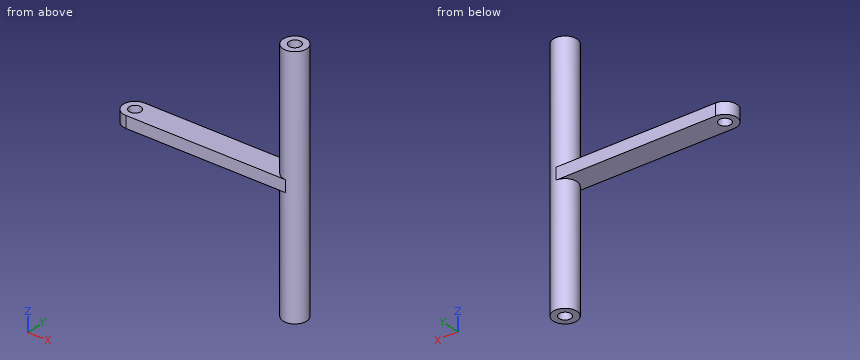
from build123d import *

# Parameters (mm, degrees)
SKETCH_1_R               = 5
SKETCH_1_R_2             = 4.376095709
EXTRUDE_1_DEPTH          = 10
SKETCH_2_R               = 10
EXTRUDE_2_DEPTH          = 100
EXTRUDE_START            = 100
SKETCH_3_R               = 10
EXTRUDE_3_DEPTH          = 100
CUT_EXTRUDE_1_DEPTH      = 224.769799627
CUT_EXTRUDE_1_DEPTH_BACK = 224.769799627
SKETCH_4_R               = 5


with BuildPart() as part:
    # 草图1 → 凸台-拉伸1 (new body)
    with BuildSketch(Plane.XY):
        with BuildLine():
            Line((-66.635, 10), (66.635, 10))
            ThreePointArc((66.635, 10), (76.635, 0), (66.635, -10))
            Line((66.635, -10), (-66.635, -10))
            ThreePointArc((-66.635, -10), (-76.635, 0), (-66.635, 10))
        make_face()
        with Locations((-66.635, 0)):
            Circle(SKETCH_1_R, mode=Mode.SUBTRACT)
        with Locations((66.635, 0)):
            Circle(SKETCH_1_R_2, mode=Mode.SUBTRACT)
    extrude(amount=EXTRUDE_1_DEPTH)

    # 草图2 → 凸台-拉伸2 (add)
    with BuildSketch(Plane.XY.offset(10)):
        with Locations(Location((66.635, 0, 0), (0, 0, 90))):
            Circle(SKETCH_2_R)
    extrude(amount=EXTRUDE_2_DEPTH)

    # 草图3 → 凸台-拉伸3 (add)
    with BuildSketch(Plane(origin=(0, 0, 0), x_dir=(-1, 0, 0), z_dir=(0, 0, -1)).offset(EXTRUDE_START)):
        with Locations((-66.635, 0)):
            Circle(SKETCH_3_R)
    extrude(amount=-EXTRUDE_3_DEPTH)

    # 草图4 → 切除-拉伸1 (cut, two sides: drawn at the far end of the back side and taken through both)
    with BuildSketch(Plane(origin=(0, 0, -100), x_dir=(-1, 0, 0), z_dir=(0, 0, -1)).offset(-CUT_EXTRUDE_1_DEPTH_BACK)):
        with Locations((-66.635, 0)):
            Circle(SKETCH_4_R)
    extrude(amount=CUT_EXTRUDE_1_DEPTH + CUT_EXTRUDE_1_DEPTH_BACK, mode=Mode.SUBTRACT)


solid = part.part
Can you work these out from the model? Positions are in its coordinate system, mm. Round coordinates to 2 decimals unless told otherwise and drop trailing zeros. Write each loop counter-clockwise with the first axis right and the second up, starting at its lowest first coordinate (ties: lowest second). Pieces come first, ordered by that corner, then holes. Notation, with made-up numbers: (-29.75, 10) -> (-15.75, 10) arc R20 cw to (-15.75, 36) -> close; hole circle Ø5 at (-15, -26.5). An arc over 180 degrees is marked (long way). Use one line per item in the form item = value. Start each with the question number.
Q1. Imagine slicing it at B-B (z = -85.5). Please give me the cut outline in (x, y) (3 decimals).
Q2. Imagine slicing it at A-A (y = 0). Please give me the cut outline in (x, z) (3 decimals).
Q3. Imagine slicing it at C-C (x = -2.5). Please give me the cut outline in (y, z).
Q4. If I drill on probe 1 along X at (y, z) = (0, 30.5) (3 decimals); probe 2 along Z at (x, y) = (32, 5.5); probe 3 along X at (y, z) = (2.5, -16.5), over which ranges is the centre line in solid material (lowest first)? Write a range as [from, to].
Q5. I'm going to push flat-ended pins straight in: P1, Ø8, axis at x = 66.635, y = 0, coming from the +Z side; P2, Ø10, axis at x = 20, y = -5, coming from the +Z side; P3, Ø3, axis at x = -58, y = -6, coming from the -Z side; P4, Ø4, axis at y = -3, z = 81, coming from the -X side. Where does each tip first touch, or does it pass through?
Worked out:
q1.outline = circle Ø20 at (66.635, 0); hole circle Ø10 at (66.635, 0)
q2.outline = (-76.635, 0) -> (-71.635, 0) -> (-71.635, 10) -> (-76.635, 10) -> close; (-61.635, 0) -> (56.635, 0) -> (56.635, -100) -> (61.635, -100) -> (61.635, 110) -> (56.635, 110) -> (56.635, 10) -> (-61.635, 10) -> close; (71.635, -100) -> (76.635, -100) -> (76.635, 110) -> (71.635, 110) -> close
q3.outline = (-10, 0) -> (10, 0) -> (10, 10) -> (-10, 10) -> close
q4.probe_1 = [56.635, 61.635], [71.635, 76.635]
q4.probe_2 = [0, 10]
q4.probe_3 = [56.95, 62.3], [70.97, 76.32]
q5.P1 = through
q5.P2 = 10
q5.P3 = 0
q5.P4 = 56.69
